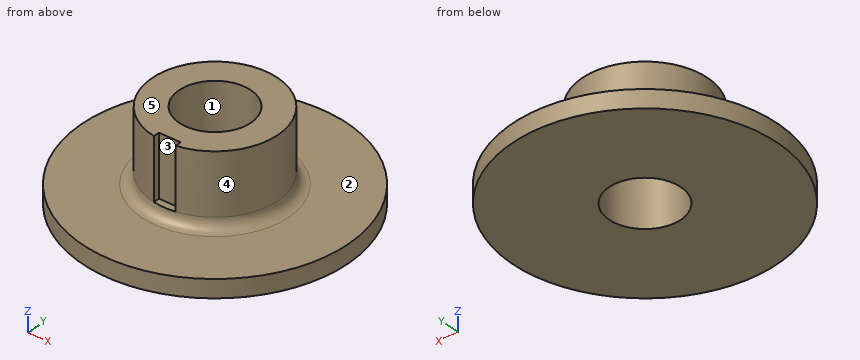
from build123d import *

# Parameters (mm, degrees)
SKETCH1_R           = 37
BOSS_EXTRUDE1_DEPTH = 5
SKETCH2_R           = 17.5
SKETCH2_R_2         = 10
BOSS_EXTRUDE2_DEPTH = 20
SKETCH3_R           = 10
CUT_EXTRUDE1_DEPTH  = 58.99137867
FILLET1_R           = 3
SKETCH4_W           = 6
SKETCH4_H           = 4
CUT_EXTRUDE2_DEPTH  = 17


with BuildPart() as part:
    # Sketch1 → Boss-Extrude1 (new body)
    with BuildSketch(Plane.XY):
        Circle(SKETCH1_R)
    extrude(amount=BOSS_EXTRUDE1_DEPTH)

    # Sketch2 → Boss-Extrude2 (add)
    with BuildSketch(Plane.XY.offset(5)):
        Circle(SKETCH2_R)
        Circle(SKETCH2_R_2, mode=Mode.SUBTRACT)
    extrude(amount=BOSS_EXTRUDE2_DEPTH)

    # Sketch3 → Cut-Extrude1 (cut, through all)
    with BuildSketch(Plane.XY.offset(25)):
        Circle(SKETCH3_R)
    extrude(amount=-CUT_EXTRUDE1_DEPTH, mode=Mode.SUBTRACT)

    # Fillet1
    fillet1_edges = [part.edges().sort_by_distance(p)[0] for p in [
        (-17.5, 0, 5),
    ]]
    fillet(fillet1_edges, radius=FILLET1_R)

    # Sketch4 → Cut-Extrude2 (cut)
    with BuildSketch(Plane.XY.offset(25)):
        with Locations((0, -17.5)):
            Rectangle(SKETCH4_W, SKETCH4_H)
    extrude(amount=-CUT_EXTRUDE2_DEPTH, mode=Mode.SUBTRACT)


solid = part.part
Verification items for the finished model (mm, model axes). Face numbers are marked on the shaded views. A direction names the side the tool comes from. Coordinates: 2 decimals unless noted, no trailing zeros. Loops run counter-clockwise (first coordinate to the right, second up) from the corner with the lowest first, then second, coordinate; pieces in that order, holes last. Notation, with made-up numbers: (44.5, 38) -> (64.5, 38) arc R8 cw to (64.5, 47) -> close; hole circle Ø6 at (47.25, 51). An arc over 180 degrees is marked (long way). Write each question's results on one line, items separated by ' | '.
Item 1: Section check D-D, the plane x = 30. Enter the section's corners in (y, z).
Found:
outline: (-21.66, 0) -> (21.66, 0) -> (21.66, 5) -> (-21.66, 5) -> close
Item 2: Section check C-C, the plane z = 13. Enter the section's corners in (x, y).
Found:
outline: (-3, -17.24) -> (-3, -15.5) -> (3, -15.5) -> (3, -17.24) arc R17.5 ccw (long way) to start; hole circle Ø20 at (0, 0)
Item 3: Mould release check, pull along X, two halves, no side actions. Record for the marked faces 3, 4 and 5: +X half, -X half, draft (parallel to the pull), parting line (faces both ways), or undercut.
Found:
face 3: undercut | face 4: parting line | face 5: draft
Item 4: Material ranges on L1, parallel to Y at x = 0, z = 13.25; L2, parallel to Z at x = -19, y = 11; L3, parallel to Y at x = -6.5, z = 2.5, recorded low to high.
Found:
L1: y = -15.5 to -10, 10 to 17.5 | L2: z = 0 to 5 | L3: y = -36.42 to -7.6, 7.6 to 36.42
Item 5: Section check B-B, the plane y = 0. Enter the section's corners in (x, z).
Found:
outline: (-37, 0) -> (-10, 0) -> (-10, 25) -> (-17.5, 25) -> (-17.5, 8) arc R3 cw to (-20.5, 5) -> (-37, 5) -> close; (10, 0) -> (37, 0) -> (37, 5) -> (20.5, 5) arc R3 cw to (17.5, 8) -> (17.5, 25) -> (10, 25) -> close
Item 6: Gauge pin test, flat ends, axial feed: pin 1 (1 mm diameter, centred on x = -0.5, y = -16.5, fed in from +Z); pin 2 (1 mm diameter, centred on x = -7, y = 29, fed in from +Z); pin 3 (4 mm diameter, centred on x = -1.5, z = 21, fed in from -Y). Record the tip position at first contact, or that the pin passes through.
Found:
pin 1: stops at z = 8 | pin 2: stops at z = 5 | pin 3: stops at y = -17.24
Item 7: Section check A-A, the plane x = 0. Enter the section's corners in (y, z).
Found:
outline: (-37, 0) -> (-10, 0) -> (-10, 25) -> (-15.5, 25) -> (-15.5, 8) -> (-17.5, 8) arc R3 cw to (-20.5, 5) -> (-37, 5) -> close; (10, 0) -> (37, 0) -> (37, 5) -> (20.5, 5) arc R3 cw to (17.5, 8) -> (17.5, 25) -> (10, 25) -> close
Item 8: Tool access check on the marked faces 1 and 2. Record the directions out of +Z, -Z, +X, -X, +Y, -Y that give a thin tool (end or side, any length) a straight path to the whole face; none if there is none.
Found:
face 1: +Z, -Z | face 2: +Z
